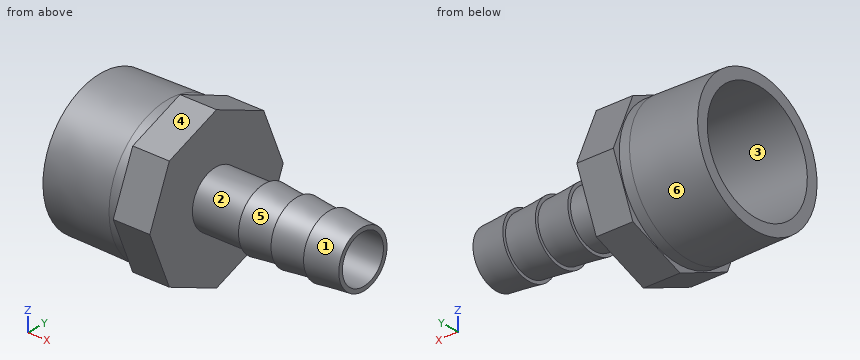
from build123d import *

# Parameters (mm, degrees)
SKETCH4_R           = 17
BOSS_EXTRUDE1_DEPTH = 9


with BuildPart() as part:
    # Sketch1 → Revolve1 (revolve)
    with BuildSketch(Plane.XY, mode=Mode.PRIVATE) as revolve1_sk:
        Polygon((19, 17), (19, 17.25), (28, 17.25), (28, 6.75), (40, 6.75), (40, 7.5), (48, 6.75), (48, 7.5), (56, 6.75), (56, 7.5), (64, 6.75), (64, 5.75), (26, 5.75), (26, 14), (0, 14), (0, 16.711991429), (16.5, 17), align=None)
    revolve(revolve1_sk.sketch.rotate(Axis((0, 0, 0), (1, 0, 0)), 90), axis=Axis((0, 0, 0), (1, 0, 0)))

    # Sketch4 → Boss-Extrude1 (add)
    with BuildSketch(Plane(origin=(28, 0, 0), x_dir=(0, 0, -1), z_dir=(1, 0, 0))):
        Polygon((0, 18.671265455), (-13.202578417, 13.202578417), (-18.671265455, 0), (-13.202578417, -13.202578417), (0, -18.671265455), (13.202578417, -13.202578417), (18.671265455, 0), (13.202578417, 13.202578417), align=None)
        with Locations(Location((0, 0, 0), (0, 0, 180))):
            Circle(SKETCH4_R, mode=Mode.SUBTRACT)
    extrude(amount=-BOSS_EXTRUDE1_DEPTH)


solid = part.part
Source: CAD feature listing. Evaluate the final solid. Frame: model axes, mm. Face numbers are marked on the shaded views. A direction names the side the tool comes from. Give positions to 0.01 mm unless a question says otherwise; leave off trailing zeros. Write each loop counter-clockwise with the first axis right and the second up, starting at its lowest first coordinate (ties: lowest second). Pieces come first, ordered by that corner, then holes. Notation, with made-up numbers: M 72,55.5 L 121,55.5 A18 ccw 121,76.5 Z; hole C 21.5,-0.5 d8. An arc over 180 degrees is marked long. Return JSON: item names as keys, results as strings. Group by question number.
1) Pin query (flat end, axial travel): P1, Ø10.5, axis at y = 0, z = 0, coming from the -X side; P2, Ø12, axis at y = -3, z = -1, coming from the -X side; P3, Ø10, axis at x = 7.5, y = 8, coming from the -Z side; P4, Ø5, axis at x = 43, y = 0, coming from the -Z side. Return the tip coordinate at first contact, or that it passes through.
2) Set-up query: the marked faces 4, 5 and 6. Return all of +Z, -Z, +X, -X, +Y, -Y with unobstructed straight access to the full face (end or side cutting, diameter ignored); none if empty.
3) Cut plane A-A, the plane x = 24. Output: boundary loops of the cut face in (y, z).
4) Cut plane B-B, the plane x = 31.5. Output: boundary loops of the cut face in (y, z).
5) Pull-direction query (X, two-part tool) for the marked faces 1, 2 and 3; classes: pulls with the +X half, pulls with the -X half, needs draft (parallel to the pull), parting line crosses it, or undercut.
6) Material intervals for line 1 along Y through (x, z) = (34, 0); line 2 along X through (y, z) = (9, 12); line 3 along X through (y, z) = (1, 9.5), sorted ascending. Write a range as [from, to].
Recorded:
{
 "1": {"P1": "passes through", "P2": "stops at x = 26", "P3": "stops at z = -16.58", "P4": "stops at z = -7.45"},
 "2": {"face 4": "+Z, +X, -X, -Y", "face 5": "none", "face 6": "-X"},
 "3": {"outline": "M -18.67,0 L -13.2,-13.2 L 0,-18.67 L 13.2,-13.2 L 18.67,0 L 13.2,13.2 L 0,18.67 L -13.2,13.2 Z; hole C 0,0 d28"},
 "4": {"outline": "C 0,0 d13.5; hole C 0,0 d11.5"},
 "5": {"face 1": "pulls with the +X half", "face 2": "undercut", "face 3": "needs draft"},
 "6": {"line 1": "y = [-6.75, -5.75], [5.75, 6.75]", "line 2": "x = [0, 28]", "line 3": "x = [26, 28]"}
}
